Geometry: final body of the model. Coordinates: model frame, mm. A direction names the side the tool comes from. Give positions to 0.01 mm unless a question says otherwise; leave off trailing zeros. Order: outer loops, then holes, each group sorted by start corner. A loop starts at its lowest first (then second) coordinate and runs counter-clockwise, first axis right, second up. Notation, with made-up numbers: (21, 59.25) -> (59, 59.25) arc R27 ccw to (59, 83.25) -> close; hole circle Ø11 at (50, -4.75). An arc over 180 degrees is marked (long way). One line per item, written item: value. Start each with the question number.
```python
from build123d import *

# Parameters (mm, degrees)
BASE_PLATE_SKETCH_W     = 135
BASE_PLATE_SKETCH_H     = 90
BASE_PLATE_DEPTH        = 24
LUG_1_DEPTH             = 10
LUG_1_BOSS_SKETCH_R     = 20
LUG_1_PIVOT_BOSS_DEPTH  = 12.5
LUG_2_DEPTH             = 10
LUG_2_BOSS_SKETCH_R     = 20
LUG_2_PIVOT_BOSS_DEPTH  = 12.5
PIVOT_HOLE_SKETCH_R     = 8
PIVOT_HOLE_16_DEPTH     = 238.407720253
MOUNTING_HOLES_SKETCH_R = 7.5
MOUNTING_HOLES_2X_DEPTH = 247.94927469


with BuildPart() as part:
    # Base Plate Sketch → Base Plate (new body)
    with BuildSketch(Plane.XY):
        with Locations((67.5, 45)):
            Rectangle(BASE_PLATE_SKETCH_W, BASE_PLATE_SKETCH_H)
    extrude(amount=-BASE_PLATE_DEPTH)

    # Lug 1 Profile → Lug 1 (add)
    with BuildSketch(Plane(origin=(90, 0, 0), x_dir=(0, 0, -1), z_dir=(1, 0, 0))):
        with BuildLine():
            Line((0, 90), (0, 180))
            ThreePointArc((0, 180), (20, 160), (40, 180))
            Line((40, 180), (76.525653448, 63))
            Line((76.525653448, 63), (36, 0))
            Line((36, 0), (24, 0))
            Line((24, 0), (24, 90))
            Line((24, 90), (0, 90))
        make_face()
    extrude(amount=-LUG_1_DEPTH)

    # Lug 1 Boss Sketch → Lug 1 Pivot Boss (add, symmetric)
    with BuildSketch(Plane(origin=(90, 0, 0), x_dir=(0, 0, -1), z_dir=(1, 0, 0))):
        with Locations((20, 180)):
            Circle(LUG_1_BOSS_SKETCH_R)
    extrude(amount=LUG_1_PIVOT_BOSS_DEPTH, both=True)

    # Lug 2 Profile → Lug 2 (add)
    with BuildSketch(Plane.ZY.offset(-45)):
        with BuildLine():
            Line((-24, 0), (-36, 0))
            Line((-36, 0), (-76.525653448, 63))
            Line((-76.525653448, 63), (-40, 180))
            ThreePointArc((-40, 180), (-20, 160), (0, 180))
            Line((0, 180), (0, 90))
            Line((0, 90), (-24, 90))
            Line((-24, 90), (-24, 0))
        make_face()
    extrude(amount=LUG_2_DEPTH)

    # Lug 2 Boss Sketch → Lug 2 Pivot Boss (add, symmetric)
    with BuildSketch(Plane.ZY.offset(-35)):
        with Locations(Location((-20, 180, 0), (0, 0, 180))):
            Circle(LUG_2_BOSS_SKETCH_R)
    extrude(amount=LUG_2_PIVOT_BOSS_DEPTH, both=True)

    # Pivot Hole Sketch → Pivot Hole Ø16 (cut, through all)
    with BuildSketch(Plane(origin=(102.5, 0, 0), x_dir=(0, 0, -1), z_dir=(1, 0, 0))):
        with Locations(Location((20, 180, 0), (0, 0, 180))):
            Circle(PIVOT_HOLE_SKETCH_R)
    extrude(amount=-PIVOT_HOLE_16_DEPTH, mode=Mode.SUBTRACT)

    # Mounting Holes Sketch → Mounting Holes 2x (cut, through all)
    with BuildSketch(Plane(origin=(0, 0, -24), x_dir=(-1, 0, 0), z_dir=(0, 0, -1))):
        with Locations((-113, 50)):
            Circle(MOUNTING_HOLES_SKETCH_R)
        with Locations((-22, 50)):
            Circle(MOUNTING_HOLES_SKETCH_R)
    extrude(amount=-MOUNTING_HOLES_2X_DEPTH, mode=Mode.SUBTRACT)


solid = part.part
```
1. Cut plane C-C, the plane x = 27. Return loops of the section in (y, z).
2. Draft query along X for faces 5 (the flat face through (67, 71, 0)), 6 (the flat face through (45, 91, -38)), 7 (the flat face through (22.5, 180, -29)). Return one class per face: pulls with the +X half, pulls with the -X half, needs draft (parallel to the pull), parting line crosses it, or undercut.
3. Pin query (flat end, axial travel): P1, Ø1, axis at x = 85.5, y = 58, coming from the -Z side; P2, Ø10, axis at x = 43.5, z = -37, coming from the +Y side; P3, Ø7, axis at x = 23.5, z = -12, coming from the +Y side. Return the tip coordinate at first contact, or that it passes through.
4. Access query for faces 1 (the flat face through (102.5, 180, -29)), 2 (the flat face through (17, 90, -12)), 3 (the flat face through (62, 46, -24)), 4 (the flat face through (47.5, 180, -29)). Directions: +Z, -Z, +X, -X, +Y, -Y. A direction counts if a zero-diameter tool reaches every point of the face in a straight line with its end or side. Return the directions, or none.
5. Cut plane D-D, the plane y = 50. Return loops of the section in (x, z).
6. Material intervals for L1, parallel to Y at x = 34.25, z = -20; L2, parallel to X at y = 123, z = -57.5; L3, parallel to Y at x = 22, z = -10, sorted ascending. Write a range as [from, to].
7. Cut plane B-B, the plane x = 113. Return loops of the section in (y, z).
8. Cut plane A-A, the plane z = -20. State how many separate pieces and enclosed holes the cut face has, then the cut area to 3 significant figures.
Answers follow:
1. outline: (0, -24) -> (44.41, -24) -> (44.41, 0) -> (0, 0) -> close; (55.59, -24) -> (90, -24) -> (90, 0) -> (55.59, 0) -> close; circle Ø40 at (180, -20); hole circle Ø16 at (180, -20)
2. face 5: needs draft
2. face 6: undercut
2. face 7: pulls with the -X half
3. P1: stops at z = -73.63
3. P2: stops at y = 196
3. P3: stops at y = 199.49
4. face 1: +Z, -Z, +X, +Y
4. face 2: +Z, -Z, -X
4. face 3: -Z, -Y
4. face 4: +Z, -Z, +Y
5. outline: (0, -24) -> (14.5, -24) -> (14.5, 0) -> (0, 0) -> close; (29.5, -24) -> (35, -24) -> (35, -68.16) -> (45, -68.16) -> (45, -24) -> (80, -24) -> (80, -68.16) -> (90, -68.16) -> (90, -24) -> (105.5, -24) -> (105.5, 0) -> (29.5, 0) -> close; (120.5, -24) -> (135, -24) -> (135, 0) -> (120.5, 0) -> close
6. L1: y = [0, 90], [160, 172], [188, 200]
6. L2: x = [35, 45], [80, 90]
6. L3: y = [0, 42.5], [57.5, 90]
7. outline: (0, -24) -> (42.5, -24) -> (42.5, 0) -> (0, 0) -> close; (57.5, -24) -> (90, -24) -> (90, 0) -> (57.5, 0) -> close
8. separate pieces: 3
8. enclosed holes: 2
8. area: 14,400 mm²
